Read the model definition and answer for the solid it produces. Units are mm, in the model's axes. Give positions to 0.01 mm unless a question says otherwise; leave off trailing zeros. Loops run counter-clockwise (first coordinate to the right, second up) from the corner with the lowest first, then second, coordinate; pieces in that order, holes last. Notation, with made-up numbers: (74, 64.5) - (107, 64.5) arc R22 ccw to (107, 102.5) - close; hole circle Ø6 at (-29, 20.25). An arc over 180 degrees is marked (long way). Put each result on its own line as item: value. Start each with the question number.
1. Consider L1, parallel to Y at x = 25, z = 2; L2, parallel to X at y = 35, z = 5.75; L3, parallel to Y at x = 28.5, z = 1.75. Determine where each line is inside the solid, lowest interval first. Write a range as from..to.
2. A cutting plane is placed at B-B, the plane x = 25. Determine the outline of the cut face in (y, z).
3. A cutting plane is placed at A-A, the plane y = 225. Determine the outline of the cut face in (x, z).
4. A cutting plane is placed at C-C, the plane z = 5. Determine the outline of the cut face in (x, y), plus the area to 3 significant figures.
5. Given pin 1 Ø16 at (x, y) = (25, 225) entering from -Z, flat-ended and moving along its own axis, determine where the tip first touches the part or whether it passes through.
6. For a pull along Y with two mould halves and no side action, classify faces 1 (the flat face through (25, 450, 5)), 2 (the flat face through (14, 228, 10)), 3 (the cylindrical face through (23.92, 410.32, 4.93)), 4 (the cylindrical face through (29, 37.8, 4.9)) as released by +Y, released by -Y, zero draft, split by the parting line, or undercut.
```python
from build123d import *

# Parameters (mm, degrees)
SKETCH_1_W      = 50
SKETCH_1_H      = 450
SKETCH_1_R      = 10
SKETCH_1_R_2    = 5
EXTRUDE_1_DEPTH = 10


with BuildPart() as part:
    # 草图1 → 凸台-拉伸1 (new body)
    with BuildSketch(Plane.XY):
        with Locations((25, 225)):
            Rectangle(SKETCH_1_W, SKETCH_1_H)
        with Locations((25, 225)):
            Circle(SKETCH_1_R, mode=Mode.SUBTRACT)
        with Locations((25, 415.201191985)):
            Circle(SKETCH_1_R_2, mode=Mode.SUBTRACT)
        with Locations(Location((25, 34.798808015, 0), (0, 0, 180))):
            Circle(SKETCH_1_R_2, mode=Mode.SUBTRACT)
    extrude(amount=EXTRUDE_1_DEPTH)


solid = part.part
```
Return value:
1. L1: y = 0..29.8, 39.8..215, 235..410.2, 420.2..450
1. L2: x = 0..20, 30..50
1. L3: y = 0..31.23, 38.37..215.63, 234.37..411.63, 418.77..450
2. outline: (0, 0) - (29.8, 0) - (29.8, 10) - (0, 10) - close; (39.8, 0) - (215, 0) - (215, 10) - (39.8, 10) - close; (235, 0) - (410.2, 0) - (410.2, 10) - (235, 10) - close; (420.2, 0) - (450, 0) - (450, 10) - (420.2, 10) - close
3. outline: (0, 0) - (15, 0) - (15, 10) - (0, 10) - close; (35, 0) - (50, 0) - (50, 10) - (35, 10) - close
4. outline: (0, 0) - (50, 0) - (50, 450) - (0, 450) - close; hole circle Ø20 at (25, 225); hole circle Ø10 at (25, 34.8); hole circle Ø10 at (25, 415.2)
4. area: 22,000 mm2
5. pin 1: passes through
6. face 1: released by +Y
6. face 2: zero draft
6. face 3: undercut
6. face 4: undercut
